Can you work these out from the model? Positions are in its coordinate system, mm. Give positions to 0.01 mm unless a question says otherwise; leave off trailing zeros. Loops run counter-clockwise (first coordinate to the right, second up) from the corner with the lowest first, then second, coordinate; pieces in that order, holes last. Notation, with made-up numbers: (78.25, 88.5) -> (113.25, 88.5) arc R22 cw to (113.25, 105.5) -> close; hole circle Ø4 at (89.5, 6). An arc over 180 degrees is marked (long way). One line per question, with ' | ' between items.
from build123d import *

# Parameters (mm, degrees)
SKETCH1_R           = 160
SKETCH1_R_2         = 57
SKETCH1_R_3         = 8
BOSS_EXTRUDE1_DEPTH = 12


with BuildPart() as part:
    # Sketch1 → Boss-Extrude1 (new body)
    with BuildSketch(Plane(origin=(0, 0, 0), x_dir=(1, 0, 0), z_dir=(0, 1, 0))):
        with Locations(Location((0, 0, 0), (0, 0, 270))):
            Circle(SKETCH1_R)
        with Locations(Location((0, 0, 0), (0, 0, 270))):
            Circle(SKETCH1_R_2, mode=Mode.SUBTRACT)
        with Locations(Location((0, 140, 0), (0, 0, 270))):
            Circle(SKETCH1_R_3, mode=Mode.SUBTRACT)
        with Locations(Location((89.990265356, 107.246222037, 0), (0, 0, 270))):
            Circle(SKETCH1_R_3, mode=Mode.SUBTRACT)
        with Locations(Location((137.873085422, 24.310744873, 0), (0, 0, 270))):
            Circle(SKETCH1_R_3, mode=Mode.SUBTRACT)
        with Locations(Location((121.24355653, -70, 0), (0, 0, 270))):
            Circle(SKETCH1_R_3, mode=Mode.SUBTRACT)
        with Locations(Location((47.882820066, -131.55696691, 0), (0, 0, 270))):
            Circle(SKETCH1_R_3, mode=Mode.SUBTRACT)
        with Locations(Location((-47.882820066, -131.55696691, 0), (0, 0, 270))):
            Circle(SKETCH1_R_3, mode=Mode.SUBTRACT)
        with Locations(Location((-121.24355653, -70, 0), (0, 0, 270))):
            Circle(SKETCH1_R_3, mode=Mode.SUBTRACT)
        with Locations(Location((-137.873085422, 24.310744873, 0), (0, 0, 270))):
            Circle(SKETCH1_R_3, mode=Mode.SUBTRACT)
        with Locations(Location((-89.990265356, 107.246222037, 0), (0, 0, 270))):
            Circle(SKETCH1_R_3, mode=Mode.SUBTRACT)
    extrude(amount=BOSS_EXTRUDE1_DEPTH)


solid = part.part
Q1. If we section it at B-B (x = 0): Write out the boundary of the cut face in (y, z), plus the area to 3 significant figures.
Entries:
outline: (0, -160) -> (12, -160) -> (12, -148) -> (0, -148) -> close; (0, -132) -> (12, -132) -> (12, -57) -> (0, -57) -> close; (0, 57) -> (12, 57) -> (12, 160) -> (0, 160) -> close | area: 2,280 mm²
Q2. If we section it at A-A (z = 0): Write out the boundary of the cut face in (x, y).
Entries:
outline: (-160, 0) -> (-57, 0) -> (-57, 12) -> (-160, 12) -> close; (57, 0) -> (160, 0) -> (160, 12) -> (57, 12) -> close
Q3. If we section it at D-D (z = 70): Write out the boundary of the cut face in (x, y).
Entries:
outline: (-143.87, 0) -> (-129.24, 0) -> (-129.24, 12) -> (-143.87, 12) -> close; (-113.24, 0) -> (113.24, 0) -> (113.24, 12) -> (-113.24, 12) -> close; (129.24, 0) -> (143.87, 0) -> (143.87, 12) -> (129.24, 12) -> close
Q4. For pin 1 Ø3 at (x, y) = (7, 10) entering from +Z; pin 2 Ø14.5 at (x, z) = (-89.99, -107.25) entering from +Y; pin 3 Ø4 at (y, z) = (6.5, 120) entering from -X, each with a flat end and sliding along its axis, tell me the tip position at first contact or that it passes through.
Entries:
pin 1: z = 159.91 | pin 2: through | pin 3: x = -108.06
Q5. If we section it at C-C (y = 9): State how many separate pieces and enclosed holes the cut face has, plus the area to 3 significant figures.
Entries:
separate pieces: 1 | enclosed holes: 10 | area: 68,400 mm²
Q6. If I drill on probe 1 along Z at (x, y) = (-42.5, 9.5); probe 2 along X at (y, z) = (10.75, -19); probe 3 along X at (y, z) = (9.25, 2.5), over which ranges is the centre line in solid material (lowest first)? Write a range as from..to.
Entries:
probe 1: -154.25..-37.98, 37.98..125.64, 137.48..154.25 | probe 2: -158.87..-143.86, -131.89..-53.74, 53.74..131.89, 143.86..158.87 | probe 3: -159.98..-56.95, 56.95..159.98
Q7. If we mould it in two halves opening along Z, with no side actions, what happens to faces 1 (the face through (145.8, 5.9, -25.4)), 2 (the face through (2, 12, 69)), 3 (the face through (-156.195, 5.916, -34.685))? For each: pulls with the +Z half, pulls with the -Z half, needs draft (parallel to the pull), parting line crosses it, or undercut.
Entries:
face 1: undercut | face 2: needs draft | face 3: parting line crosses it
